The model under review builds one solid part; all positions refer to its coordinate system, in mm. A direction names the side the tool comes from. Give positions to 0.01 mm unless a question says otherwise; leave off trailing zeros. Loops run counter-clockwise (first coordinate to the right, second up) from the corner with the lowest first, then second, coordinate; pieces in that order, holes last. Notation, with made-up numbers: M 21,33 L 45,33 A9 ccw 45,42 Z; hole C -31.5,12 d9. An arc over 180 degrees is marked long. Put each result on its own line as item: value. Start each with the question number.
from build123d import *

# Parameters (mm, degrees)
SKETCH1_W           = 260
SKETCH1_H           = 196
SKETCH1_W_2         = 220
SKETCH1_H_2         = 156
BOSS_EXTRUDE1_DEPTH = 5
FILLET1_R           = 5
FILLET2_R           = 10


with BuildPart() as part:
    # Sketch1 → Boss-Extrude1 (new body)
    with BuildSketch(Plane.XY):
        Rectangle(SKETCH1_W, SKETCH1_H)
        Rectangle(SKETCH1_W_2, SKETCH1_H_2, mode=Mode.SUBTRACT)
    extrude(amount=BOSS_EXTRUDE1_DEPTH)

    # Fillet1
    fillet1_edges = [part.edges().sort_by_distance(p)[0] for p in [
        (-130, 98, 2.5),
        (130, 98, 2.5),
        (130, -98, 2.5),
        (-130, -98, 2.5),
    ]]
    fillet(fillet1_edges, radius=FILLET1_R)

    # Fillet2
    fillet2_edges = [part.edges().sort_by_distance(p)[0] for p in [
        (-110, 78, 2.5),
        (-110, -78, 2.5),
        (110, -78, 2.5),
        (110, 78, 2.5),
    ]]
    fillet(fillet2_edges, radius=FILLET2_R)


solid = part.part
(1) We need section C-C, the plane x = 6.5. Write out the cut boundary in (y, z).
(2) For faces 5 (the flat face through (130, -1, 2)), 6 (the cylindrical face through (106.99, -75.15, 2.54)), list the 3-axis set-ups (+Z, -Z, +X, -X, +Y, -Y) from which the entire face can be reached by the end or side of a thin tool; tool diameter is ignored.
(3) To check wall thickness, follow L1, parallel to X at y = -53, z = 0.45; L2, parallel to Y at x = -78.5, z = 4.55. State the ranges of each line that lie inside material, in increasing order. Write a range as [from, to].
(4) We need section B-B, the plane y = -24. Write out the cut boundary in (x, z).
(5) We need section A-A, the plane z = 2.4. Write out the cut boundary in (x, y).
(6) Draft analysis for pull direction X (two halves, no side actions). For faces 1 (the flat face through (-1, 78, 2)), 2 (the cylindrical face through (128, 97, 3)), 3 (the flat face through (-130, -1, 2)), 4 (the flat face through (-2, -86, 5)), state which applies: +X half, -X half, draft (parallel to the pull), parting line (faces both ways), or undercut.
Check sheet entries:
1. outline: M -98,0 L -78,0 L -78,5 L -98,5 Z; M 78,0 L 98,0 L 98,5 L 78,5 Z
2. face 5: +Z, -Z, +X, +Y, -Y
2. face 6: +Z, -Z
3. L1: x = [-130, -110], [110, 130]
3. L2: y = [-98, -78], [78, 98]
4. outline: M -130,0 L -110,0 L -110,5 L -130,5 Z; M 110,0 L 130,0 L 130,5 L 110,5 Z
5. outline: M -130,-93 A5 ccw -125,-98 L 125,-98 A5 ccw 130,-93 L 130,93 A5 ccw 125,98 L -125,98 A5 ccw -130,93 Z; hole M -110,-68 A10 ccw -100,-78 L 100,-78 A10 ccw 110,-68 L 110,68 A10 ccw 100,78 L -100,78 A10 ccw -110,68 Z
6. face 1: undercut
6. face 2: +X half
6. face 3: -X half
6. face 4: draft
